from build123d import *

# Parameters (mm, degrees)
SKETCH1_R           = 1
BOSS_EXTRUDE1_DEPTH = 13
SKETCH2_W           = 2.556803996
SKETCH2_H           = 0.5
CUT_EXTRUDE1_DEPTH  = 2


with BuildPart() as part:
    # Sketch1 → Boss-Extrude1 (new body)
    with BuildSketch(Plane(origin=(0, 0, 0), x_dir=(0, 0, -1), z_dir=(1, 0, 0))):
        with Locations(Location((0, 0, 0), (0, 0, 180))):
            Circle(SKETCH1_R)
    extrude(amount=BOSS_EXTRUDE1_DEPTH)

    # Sketch2 → Cut-Extrude1 (cut)
    with BuildSketch(Plane(origin=(13, 0, 0), x_dir=(0, 0, -1), z_dir=(1, 0, 0))):
        Rectangle(SKETCH2_W, SKETCH2_H)
    extrude(amount=-CUT_EXTRUDE1_DEPTH, mode=Mode.SUBTRACT)


solid = part.part
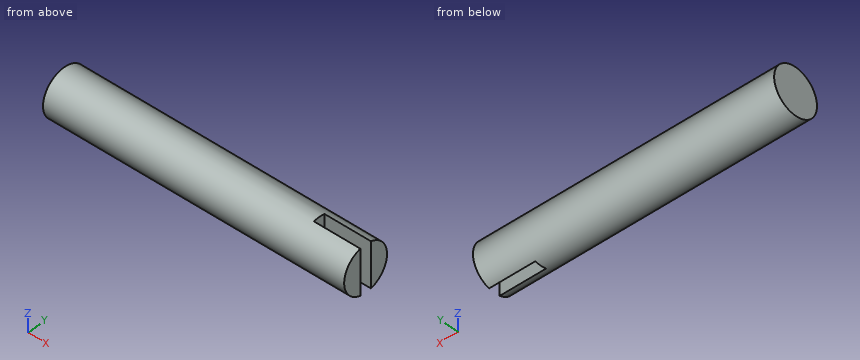
The model under review builds one solid part; all positions refer to its coordinate system, in mm. Round coordinates to 2 decimals unless told otherwise and drop trailing zeros. Loops run counter-clockwise (first coordinate to the right, second up) from the corner with the lowest first, then second, coordinate; pieces in that order, holes last. Notation, with made-up numbers: (-4.5, 11) -> (39.5, 11) arc R22 cw to (39.5, 46) -> close; hole circle Ø8 at (18.5, 72). An arc over 180 degrees is marked (long way). One line per question, with ' | ' between items. Start each with the question number.
Item 1: Wall thickness on line 1 along Y through (x, z) = (12, 0.25); line 2 along Z through (x, y) = (8.5, -0.25); line 3 along Y through (x, z) = (4, -0.05): over which ranges is each line inside the solid? List them lowest first. Write a range as [from, to].
Item 2: Add section B-B, the plane x = 12.25. Write out the cut boundary in (y, z), then the cut area to 3 significant figures.
Item 3: Add section A-A, the plane z = -0.8. Write out the cut boundary in (x, y).
Item 4: Add section C-C, the plane y = 0. Write out the cut boundary in (x, z), then the cut area to 3 significant figures.
Item 5: Add section D-D, the plane z = 0. Write out the cut boundary in (x, y).
Return value:
1) line 1: y = [-0.97, -0.25], [0.25, 0.97] | line 2: z = [-0.97, 0.97] | line 3: y = [-1, 1]
2) outline: (-0.25, -0.97) -> (-0.25, 0.97) arc R1 ccw to start; (0.25, -0.97) arc R1 ccw to (0.25, 0.97) -> close | area: 2.15 mm2
3) outline: (0, -0.6) -> (13, -0.6) -> (13, -0.25) -> (11, -0.25) -> (11, 0.25) -> (13, 0.25) -> (13, 0.6) -> (0, 0.6) -> close
4) outline: (0, -1) -> (11, -1) -> (11, 1) -> (0, 1) -> close | area: 22.0 mm2
5) outline: (0, -1) -> (13, -1) -> (13, -0.25) -> (11, -0.25) -> (11, 0.25) -> (13, 0.25) -> (13, 1) -> (0, 1) -> close
